Model file for the job. Use its own axes, mm. A direction names the side the tool comes from. Round coordinates to 2 decimals unless told otherwise and drop trailing zeros. Loops run counter-clockwise (first coordinate to the right, second up) from the corner with the lowest first, then second, coordinate; pieces in that order, holes last. Notation, with made-up numbers: (77, 5.5) -> (95, 5.5) arc R11 ccw to (95, 17.5) -> close; hole circle Ø9 at (-35, 39.25). An arc over 180 degrees is marked (long way). Use a Markdown table: item, result.
from build123d import *

# Parameters (mm, degrees)
SKETCH_1_W                   = 20
SKETCH_1_H                   = 60
EXTRUDE_1_DEPTH              = 8
SKETCH_2_W                   = 19.5
SKETCH_2_H                   = 10
CUT_EXTRUDE_1_DEPTH          = 14
CHAMFER_1_SIZE               = 3
CUT_EXTRUDE_3_DEPTH          = 36.440090293
CUT_EXTRUDE_3_DEPTH_BACK     = 36.440090293
CHAMFER_2_SIZE               = 0.5
SKETCH_6_R                   = 1.5
CUT_EXTRUDE_4_DEPTH          = 14
HOLE_WIZARD_M4_1_D           = 4.5
HOLE_WIZARD_M4_1_CBORE_D     = 8
HOLE_WIZARD_M4_1_CBORE_DEPTH = 4.4
SKETCH_11_W                  = 10
SKETCH_11_H                  = 22
CUT_EXTRUDE_7_DEPTH          = 36.440090293
SKETCH_12_W                  = 30
SKETCH_12_H                  = 6
CUT_EXTRUDE_8_DEPTH          = 37.932370625
CUT_EXTRUDE_9_DEPTH          = 34.166247904
FILLET_2_R                   = 3
SKETCH_14_W                  = 18.511605667
SKETCH_14_H                  = 56.283608206
CUT_EXTRUDE_10_DEPTH         = 36.440090293
HOLE_WIZARD_M3_1_D           = 2.5


with BuildPart() as part:
    # 草图1 → 凸台-拉伸1 (new, symmetric)
    with BuildSketch(Plane(origin=(0, 0, 0), x_dir=(1, 0, 0), z_dir=(0, 1, 0))):
        Rectangle(SKETCH_1_W, SKETCH_1_H)
    extrude(amount=EXTRUDE_1_DEPTH, both=True)

    # 草图2 → 切除-拉伸1 (cut)
    with BuildSketch(Plane(origin=(10, 0, 0), x_dir=(0, 0, -1), z_dir=(1, 0, 0))):
        with Locations((20.25, 0)):
            Rectangle(SKETCH_2_W, SKETCH_2_H)
    extrude(amount=-CUT_EXTRUDE_1_DEPTH, mode=Mode.SUBTRACT)

    # 倒角1
    chamfer_1_edges = [part.edges().sort_by_distance(p)[0] for p in [
        (10, -6.5, -30),
        (10, 6.5, -30),
    ]]
    chamfer(chamfer_1_edges, length=CHAMFER_1_SIZE)

    # 草图5 → 切除-拉伸3 (cut, two sides: drawn at the far end of the back side and taken through both)
    with BuildSketch(Plane.XZ.offset(8).offset(-CUT_EXTRUDE_3_DEPTH_BACK)):
        Polygon((-6, 164.19339757), (-6, 30), (-6, 2), (-10, -0.800830153), (-119.92479595, -77.771000913), (-362.743295595, 36.555933952), (-248.818499645, 278.520332435), align=None)
    extrude(amount=CUT_EXTRUDE_3_DEPTH + CUT_EXTRUDE_3_DEPTH_BACK, mode=Mode.SUBTRACT)

    # 倒角2
    chamfer_2_edges = [part.edges().sort_by_distance(p)[0] for p in [
        (-6, 0, 30),
        (10, 0, 30),
    ]]
    chamfer(chamfer_2_edges, length=CHAMFER_2_SIZE)

    # 草图6 → 切除-拉伸4 (cut)
    with BuildSketch(Plane(origin=(10, 0, 0), x_dir=(0, 0, -1), z_dir=(1, 0, 0))):
        with Locations((10.5, 5)):
            Circle(SKETCH_6_R)
        with Locations((10.5, -5)):
            Circle(SKETCH_6_R)
    extrude(amount=-CUT_EXTRUDE_4_DEPTH, mode=Mode.SUBTRACT)

    # M4 六角凹头螺钉的柱形沉头孔1 (through all)
    with Locations(Plane.ZY.offset(10)):
        with Locations((-15.500000304, 6.53e-07), (-24.500000304, 6.53e-07)):
            CounterBoreHole(HOLE_WIZARD_M4_1_D / 2, HOLE_WIZARD_M4_1_CBORE_D / 2, HOLE_WIZARD_M4_1_CBORE_DEPTH)

    # 草图11 → 切除-拉伸7 (cut, through all)
    with BuildSketch(Plane.XZ.offset(8)):
        with Locations((5, -19)):
            Rectangle(SKETCH_11_W, SKETCH_11_H)
    extrude(amount=-CUT_EXTRUDE_7_DEPTH, mode=Mode.SUBTRACT)

    # 草图12 → 切除-拉伸8 (cut, through all)
    with BuildSketch(Plane(origin=(10, 0, 0), x_dir=(0, 0, -1), z_dir=(1, 0, 0))):
        with Locations((-15, -5)):
            Rectangle(SKETCH_12_W, SKETCH_12_H)
    extrude(amount=-CUT_EXTRUDE_8_DEPTH, mode=Mode.SUBTRACT)

    # 草图13 → 切除-拉伸9 (cut, through all)
    with BuildSketch(Plane.XZ.offset(2)):
        Polygon((10, 14.214190818), (5.948732796, 20), (10, 25.785809182), align=None)
    extrude(amount=-CUT_EXTRUDE_9_DEPTH, mode=Mode.SUBTRACT)

    # 圆角2
    fillet_2_edges = [part.edges().sort_by_distance(p)[0] for p in [
        (5.948732796, 3, 20),
    ]]
    fillet(fillet_2_edges, radius=FILLET_2_R)

    # 草图14 → 切除-拉伸10 (cut, through all)
    with BuildSketch(Plane(origin=(0, 8, 0), x_dir=(1, 0, 0), z_dir=(0, 1, 0))):
        with Locations((10.255802834, -12.692083527)):
            Rectangle(SKETCH_14_W, SKETCH_14_H)
    extrude(amount=-CUT_EXTRUDE_10_DEPTH, mode=Mode.SUBTRACT)

    # M3 螺纹孔1 (through all)
    with Locations(Plane(origin=(1, 0, 0), x_dir=(0, 0, -1), z_dir=(1, 0, 0))):
        with Locations((-25.5, 3), (-14.5, 3)):
            Hole(HOLE_WIZARD_M3_1_D / 2)


solid = part.part
Q1. Tool access for faces 1 (the face through (-2, 0, -10.5)), 2 (the face through (-7.831, 0.176, -19.496)), 3 (the face through (0.5, -0.1, -8)): list every direction of +Z, -Z, +X, -X, +Y, -Y with a clear straight run to the whole face (end or side of a thin tool).
Results list:
| item | result |
|---|---|
| face 1 | -Z, +X |
| face 2 | -X |
| face 3 | -Z, +X, +Y, -Y |
Q2. Flat gauge pins, fed straight in: pin 1 (3 mm diameter, centred on x = -6, z = 21, fed in from -Y); pin 2 (8 mm diameter, centred on y = 4, z = 9.5, fed in from -X); pin 3 (4 mm diameter, centred on y = 2, z = -25.5, fed in from -X); pin 4 (1.2 mm diameter, centred on x = -2.5, y = 0.5, fed in from -Z). Where does each tip first touch, or does it go through?
Results list:
| item | result |
|---|---|
| pin 1 | stops at y = -2 |
| pin 2 | stops at x = -6 |
| pin 3 | stops at x = -10 |
| pin 4 | stops at z = -10.5 |
Q3. Band-saw the part on A-A, the plane z = -24.5. Give the cut face in (x, y), plus the area to 3 significant figures.
Results list:
| item | result |
|---|---|
| outline | (-10, -8) -> (0, -8) -> (0, -5) -> (-4, -5) -> (-4, -2.25) -> (-5.6, -2.25) -> (-5.6, -4) -> (-10, -4) -> close; (-10, 4) -> (-5.6, 4) -> (-5.6, 2.25) -> (-4, 2.25) -> (-4, 5) -> (0, 5) -> (0, 8) -> (-10, 8) -> close |
| area | 77.6 mm² |
Q4. Band-saw the part on B-B, the plane x = -3.25. Give the cut face in (y, z), plus the area to 3 significant figures.
Results list:
| item | result |
|---|---|
| outline | (-8, -30) -> (-5, -30) -> (-5, -12) arc R1.5 cw (long way) to (-3.5, -10.5) -> (3.5, -10.5) arc R1.5 cw (long way) to (5, -12) -> (5, -30) -> (8, -30) -> (8, 30) -> (-2, 30) -> (-2, 0) -> (-8, 0) -> close; hole circle Ø2.5 at (3, 14.5); hole circle Ø2.5 at (3, 25.5) |
| area | 565 mm² |
Q5. Pull direction Y, two halves, no side cores. Call faces 4 (the face through (-1.972, -6.025, -9.405)), 5 (the face through (0, -5.4, -19.2)), 6 (the face through (-5, 8, 0)): released by +Y, released by -Y, zero draft, split by the parting line, or undercut.
Results list:
| item | result |
|---|---|
| face 4 | undercut |
| face 5 | zero draft |
| face 6 | released by +Y |
Q6. Drill centre lines: L1, parallel to Y at x = -1, z = -20; L2, parallel to Z at x = 0.5, y = 2.25; L3, parallel to Y at x = -8.55, z = -24.5. Where is each one in solid material? Low to high. Write a range as from..to.
Results list:
| item | result |
|---|---|
| L1 | y = -8..-5, 5..8 |
| L2 | z = -8..13.5, 15.5..24.5, 26.5..30 |
| L3 | y = -8..-4, 4..8 |
Q7. Band-saw the part on C-C, the plane z = 25.5. Give the cut face in (x, y).
Results list:
| item | result |
|---|---|
| outline | (-6, -2) -> (1, -2) -> (1, 1.75) -> (-6, 1.75) -> close; (-6, 4.25) -> (1, 4.25) -> (1, 8) -> (-6, 8) -> close |
Q8. Band-saw the part on D-D, the plane x = -7.25. Give the cut face in (y, z).
Results list:
| item | result |
|---|---|
| outline | (-8, -30) -> (8, -30) -> (8, 1.12) -> (-2, 1.12) -> (-2, 0) -> (-8, 0) -> close; hole circle Ø8 at (0, -24.5); hole circle Ø8 at (0, -15.5) |
